Read the model definition and answer for the solid it produces. Units are mm, in the model's axes. Face numbers are marked on the shaded views. A direction names the side the tool comes from. Round coordinates to 2 decimals unless told otherwise and drop trailing zeros. Order: outer loops, then holes, each group sorted by start corner. A loop starts at its lowest first (then second) coordinate and runs counter-clockwise, first axis right, second up. Notation, with made-up numbers: M -11.5,71.5 L 21.5,71.5 A19 ccw 21.5,100.5 Z; hole C 36,23.5 d2. An arc over 180 degrees is marked long. Use one line per item in the form item = value. Start each with the question number.
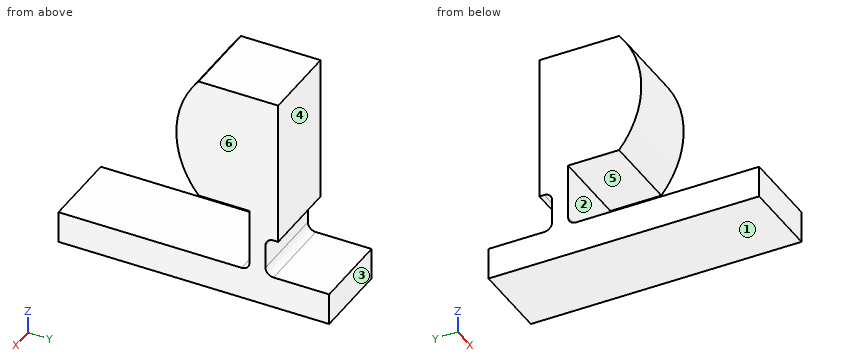
from build123d import *

# Parameters (mm, degrees)
BACK_PLATE_SKETCH_W = 20
BACK_PLATE_SKETCH_H = 170
BACK_PLATE_DEPTH    = 25
NECK_BOSS_DEPTH     = 50
NECK_FILLET_R5_R    = 5
ARM_BLOCK_DEPTH     = 50


with BuildPart() as part:
    # Back Plate Sketch → Back Plate (new, symmetric)
    with BuildSketch(Plane(origin=(0, 0, 0), x_dir=(0, 0, -1), z_dir=(1, 0, 0))):
        Rectangle(BACK_PLATE_SKETCH_W, BACK_PLATE_SKETCH_H)
    extrude(amount=BACK_PLATE_DEPTH, both=True)

    # Neck Boss Sketch → Neck Boss (add, through all)
    with BuildSketch(Plane(origin=(25, 0, 0), x_dir=(0, 0, -1), z_dir=(1, 0, 0))):
        with BuildLine():
            Line((-30, 45), (-10, 45))
            Line((-10, 45), (-10, 35))
            Line((-10, 35), (-50, 35))
            Line((-50, 35), (-50, 53))
            Line((-50, 53), (-35, 53))
            Line((-35, 53), (-35, 50))
            ThreePointArc((-35, 50), (-33.535533906, 46.464466094), (-30, 45))
        make_face()
    extrude(amount=-NECK_BOSS_DEPTH)

    # Neck Fillet R5
    neck_fillet_r5_edges = [part.edges().sort_by_distance(p)[0] for p in [
        (0, 45, 10),
        (0, 35, 10),
    ]]
    fillet(neck_fillet_r5_edges, radius=NECK_FILLET_R5_R)

    # Arm Block Sketch → Arm Block (add, through all)
    with BuildSketch(Plane(origin=(25, 0, 0), x_dir=(0, 0, -1), z_dir=(1, 0, 0))):
        with BuildLine():
            Line((-50, 53), (-50, 3))
            ThreePointArc((-50, 3), (-88.522720569, -11), (-127.045441137, 3))
            Line((-127.045441137, 3), (-127.045441137, 53))
            Line((-127.045441137, 53), (-50, 53))
        make_face()
    extrude(amount=-ARM_BLOCK_DEPTH)


solid = part.part
Item 1: Section C-C (z = 115.5) is taken. Write down the section's boundary in (x, y).
Item 2: For a pull along Z with two mould halves and no side action, classify the marked faces 1, 2 and 3 as pulls with the +Z half, pulls with the -Z half, needs draft (parallel to the pull), parting line crosses it, or undercut.
Item 3: A tool of negligible diameter and unlimited length cuts with its end or side. For the marked faces 4, 5 and 6, from which of +Z, -Z, +X, -X, +Y, -Y can it reach the whole face along a straight path? Write none if from no direction.
Item 4: Section D-D (y = -24.5) is taken. Write down the section's boundary in (x, z), and give its area (3 significant figures).
Item 5: Section A-A (y = 6) is taken. Write down the section's boundary in (x, z).
Item 6: Find the intervals of material crossed by L1, parallel to Z at x = 10, y = 65; L2, parallel to Y at x = -12.5, z = 15; L3, parallel to Z at x = 8, y = 25, in increasing order. Write a range as [from, to].
Item 7: Given P1, Ø8, axis at x = 17.5, z = 100.5, coming from the +Y side; P2, Ø6, axis at x = -2, z = 64, coming from the -Y side; P3, Ø8, axis at x = -19.5, z = 35, coming from the -Y side, each flat-ended and moving along its own axis, determine where each tip first touches the part or whether it passes through.
Item 8: Section B-B (x = -1) is taken. Write down the section's boundary in (y, z).
The answers:
q1.outline = M -25,-4.59 L 25,-4.59 L 25,53 L -25,53 Z
q2.face_1 = pulls with the -Z half
q2.face_2 = undercut
q2.face_3 = needs draft
q3.face_4 = +Z, +X, -X, +Y
q3.face_5 = +X, -X, -Y
q3.face_6 = +Z, -Z, +X, +Y, -Y
q4.outline = M -25,-10 L 25,-10 L 25,10 L -25,10 Z
q4.area = 1,000 mm²
q5.outline = M -25,-10 L 25,-10 L 25,10 L -25,10 Z; M -25,50 L 25,50 L 25,127.05 L -25,127.05 Z
q6.L1 = [-10, 10]
q6.L2 = [35, 45]
q6.L3 = [-10, 10], [50, 127.05]
q7.P1 = 53
q7.P2 = -7.01
q7.P3 = 35
q8.outline = M -85,-10 L 85,-10 L 85,10 L 50,10 A5 cw 45,15 L 45,30 A5 cw 50,35 L 53,35 L 53,127.05 L 3,127.05 A60 ccw 3,50 L 35,50 L 35,15 A5 cw 30,10 L -85,10 Z
